from build123d import *

# Parameters (mm, degrees)
CURVED_DUCT_BODY_DEPTH             = 17.5
SKETCH1_4_W                        = 50
SKETCH1_4_H                        = 5
SKETCH1_4_W_2                      = 5
SKETCH1_4_H_2                      = 50
MOUNTING_FLANGES_DEPTH             = 27.5
SKETCH1_5_W                        = 24
SKETCH1_5_H                        = 5
SKETCH1_5_W_2                      = 5
SKETCH1_5_H_2                      = 24
DUCT_RELIEF_CUT_29MM_DEPTH         = 14.5
DOWEL_HOLES_6_FLANGE_A_D           = 6
DOWEL_HOLES_6_FLANGE_A_CSINK_D     = 6.05
DOWEL_HOLES_6_FLANGE_A_CSINK_ANGLE = 90
DOWEL_HOLES_6_FLANGE_B_D           = 6
DOWEL_HOLES_6_FLANGE_B_CSINK_D     = 6.05
DOWEL_HOLES_6_FLANGE_B_CSINK_ANGLE = 90


with BuildPart() as part:
    # Bracket Profile Sketch → Curved Duct Body (new, symmetric)
    with BuildSketch(Plane.YX):
        with BuildLine():
            Line((15, 5), (15, 10))
            ThreePointArc((15, 10), (-2.573593129, 52.426406871), (-45, 70))
            Line((-45, 70), (-50, 70))
            Line((-50, 70), (-50, 40))
            Line((-50, 40), (-45, 40))
            ThreePointArc((-45, 40), (-23.786796564, 31.213203436), (-15, 10))
            Line((-15, 10), (-15, 5))
            Line((-15, 5), (15, 5))
        make_face()
    extrude(amount=CURVED_DUCT_BODY_DEPTH, both=True)

    # Sketch1_4 → Mounting Flanges (add, symmetric)
    with BuildSketch(Plane.YX):
        with Locations((0, 2.5)):
            Rectangle(SKETCH1_4_W, SKETCH1_4_H)
        with Locations((-52.5, 55)):
            Rectangle(SKETCH1_4_W_2, SKETCH1_4_H_2)
    extrude(amount=MOUNTING_FLANGES_DEPTH, both=True)

    # Sketch1_5 → Duct Relief Cut 29mm (cut, symmetric)
    with BuildSketch(Plane.YX):
        with BuildLine():
            Line((-12, 5), (12, 5))
            Line((12, 5), (12, 10))
            ThreePointArc((12, 10), (-4.694913472, 50.305086528), (-45, 67))
            Line((-45, 67), (-50, 67))
            Line((-50, 67), (-50, 43))
            Line((-50, 43), (-45, 43))
            ThreePointArc((-45, 43), (-21.665476221, 33.334523779), (-12, 10))
            Line((-12, 10), (-12, 5))
        make_face()
        with Locations((0, 2.5)):
            Rectangle(SKETCH1_5_W, SKETCH1_5_H)
        with Locations((-52.5, 55)):
            Rectangle(SKETCH1_5_W_2, SKETCH1_5_H_2)
    extrude(amount=DUCT_RELIEF_CUT_29MM_DEPTH, both=True, mode=Mode.SUBTRACT)

    # Dowel Holes _6 Flange A (through all)
    with Locations(Plane(origin=(5, 0, 0), x_dir=(0, 0, -1), z_dir=(1, 0, 0))):
        with Locations((-21, 18.5), (21, 18.5), (21, -18.5), (-21, -18.5)):
            CounterSinkHole(DOWEL_HOLES_6_FLANGE_A_D / 2, DOWEL_HOLES_6_FLANGE_A_CSINK_D / 2, counter_sink_angle=DOWEL_HOLES_6_FLANGE_A_CSINK_ANGLE)

    # Dowel Holes _6 Flange B (through all)
    with Locations(Plane(origin=(0, -50, 0), x_dir=(1, 0, 0), z_dir=(0, 1, 0))):
        with Locations((73.5, 21), (73.5, -21), (36.5, 21), (36.5, -21)):
            CounterSinkHole(DOWEL_HOLES_6_FLANGE_B_D / 2, DOWEL_HOLES_6_FLANGE_B_CSINK_D / 2, counter_sink_angle=DOWEL_HOLES_6_FLANGE_B_CSINK_ANGLE)


solid = part.part
The model under review builds one solid part; all positions refer to its coordinate system, in mm. A direction names the side the tool comes from. Coordinates: 2 decimals unless noted, no trailing zeros. Order: outer loops, then holes, each group sorted by start corner. A loop starts at its lowest first (then second) coordinate and runs counter-clockwise, first axis right, second up. Notation, with made-up numbers: (10, 79.5) -> (16, 79.5) arc R21 ccw to (16, 97.5) -> close; hole circle Ø10 at (14.25, 84). An arc over 180 degrees is marked (long way). Answer in a Markdown table with one row per item.
(1) Insertion check: pin 1 (6 mm diameter, centred on x = 25, z = 14, fed in from -Y); pin 2 (4 mm diameter, centred on x = 22, z = 16.5, fed in from +Y); pin 3 (15 mm diameter, centred on y = 7, z = 6, fed in from +X); pin 4 (3.5 mm diameter, centred on y = -18.5, z = 21, fed in from +X). Each pin has a flat end and moves straight along its axis. Give the tip position at first contact, or say it passes through.
Answers:
| item | result |
|---|---|
| pin 1 | y = -21 |
| pin 2 | y = 14.16 |
| pin 3 | x = 50.25 |
| pin 4 | through |
(2) Machinability: for faces 4 (the flat face through (7, 15, 0)), 5 (the flat face through (2, -25, 0)), 6 (the flat face through (41, -15, -14.5)), which of the approach directions +Z, -Z, +X, -X, +Y, -Y give a long, thin tool a straight path to every point of the face, cutting with its end or side? Answer none if there is none.
Answers:
| item | result |
|---|---|
| face 4 | +Z, -Z, +X, +Y |
| face 5 | +Z, -Z, -X, -Y |
| face 6 | none |
(3) Wall thickness on line 1 along X through (y, z) = (-53.7, -21); line 2 along Z through (x, y) = (2.7, 18.5); line 3 along Y through (x, z) = (2, 21): over which ranges is each line inside the solid? List them lowest first.
Answers:
| item | result |
|---|---|
| line 1 | 30 to 33.5, 39.5 to 70.5, 76.5 to 80 |
| line 2 | -27.5 to -24, -18 to 18, 24 to 27.5 |
| line 3 | -25 to -21.5, -15.5 to 15.5, 21.5 to 25 |
(4) The part is to be moulded in two halves that separate along Y. For faces 1 (the cylindrical face through (2.5, 16.7, 18.6)), 2 (the flat face through (71, -55, 0)), 3 (the flat face through (0, 16, 0)), say which applies: +Y half, -Y half, draft (parallel to the pull), parting line (faces both ways), or undercut.
Answers:
| item | result |
|---|---|
| face 1 | undercut |
| face 2 | -Y half |
| face 3 | draft |
(5) Consider section B-B (x = 36.5). Write out the cut boundary in (y, z) (3 decimals), plus the area to 3 significant figures.
Answers:
| item | result |
|---|---|
| outline | (-55, -27.5) -> (-50, -27.5) -> (-50, -24.025) -> (-50.025, -24) -> (-55, -24) -> close; (-55, -18) -> (-50.025, -18) -> (-50, -17.975) -> (-50, 17.975) -> (-50.025, 18) -> (-55, 18) -> close; (-55, 24) -> (-50.025, 24) -> (-50, 24.025) -> (-50, 27.5) -> (-55, 27.5) -> close; (-30.938, -17.5) -> (8.831, -17.5) -> (8.831, 17.5) -> (-30.938, 17.5) -> close; hole (-25.334, -14.5) -> (5.465, -14.5) -> (5.465, 14.5) -> (-25.334, 14.5) -> close |
| area | 714 mm² |
(6) Consider section D-D (z = 0.5). Write out the cut boundary in (x, y), plus the area to 3 significant figures.
Answers:
| item | result |
|---|---|
| outline | (0, -25) -> (5, -25) -> (5, -15) -> (10, -15) arc R30 cw to (40, -45) -> (40, -50) -> (30, -50) -> (30, -55) -> (43, -55) -> (43, -45) arc R33 ccw to (10, -12) -> (0, -12) -> close; (0, 12) -> (10, 12) arc R57 cw to (67, -45) -> (67, -55) -> (80, -55) -> (80, -50) -> (70, -50) -> (70, -45) arc R60 ccw to (10, 15) -> (5, 15) -> (5, 25) -> (0, 25) -> close |
| area | 744 mm² |
(7) Consider section A-A (z = -21). State how many separate pieces and enclosed holes the cut face has, plus the area to 3 significant figures.
Answers:
| item | result |
|---|---|
| separate pieces | 6 |
| enclosed holes | 0 |
| area | 380 mm² |
(8) Consider section C-C (y = -18.5). Write out the cut boundary in (x, z) (3 decimals).
Answers:
| item | result |
|---|---|
| outline | (0, -27.5) -> (5, -27.5) -> (5, -24.025) -> (4.975, -24) -> (0, -24) -> close; (0, -18) -> (4.975, -18) -> (5, -17.975) -> (5, 17.975) -> (4.975, 18) -> (0, 18) -> close; (0, 24) -> (4.975, 24) -> (5, 24.025) -> (5, 27.5) -> (0, 27.5) -> close; (24.062, -17.5) -> (63.831, -17.5) -> (63.831, 17.5) -> (24.062, 17.5) -> close; hole (29.666, -14.5) -> (60.465, -14.5) -> (60.465, 14.5) -> (29.666, 14.5) -> close |
